Part print with two shaded views. Sizes in mm from the minimum x, y, z corner. A direction names the side the tool comes from. Coordinates: 2 decimals unless noted, no trailing zeros. Loops run counter-clockwise (first coordinate to the right, second up) from the corner with the lowest first, then second, coordinate; pieces in that order, holes last. Notation, with made-up numbers: M -37.75,-23.75 L 2.25,-23.75 A23 cw 2.25,6.25 Z; hole C 17,15 d4. An arc over 180 degrees is marked long. Use CSV: the item, a comma, the result in double quotes. Start each with the question number.
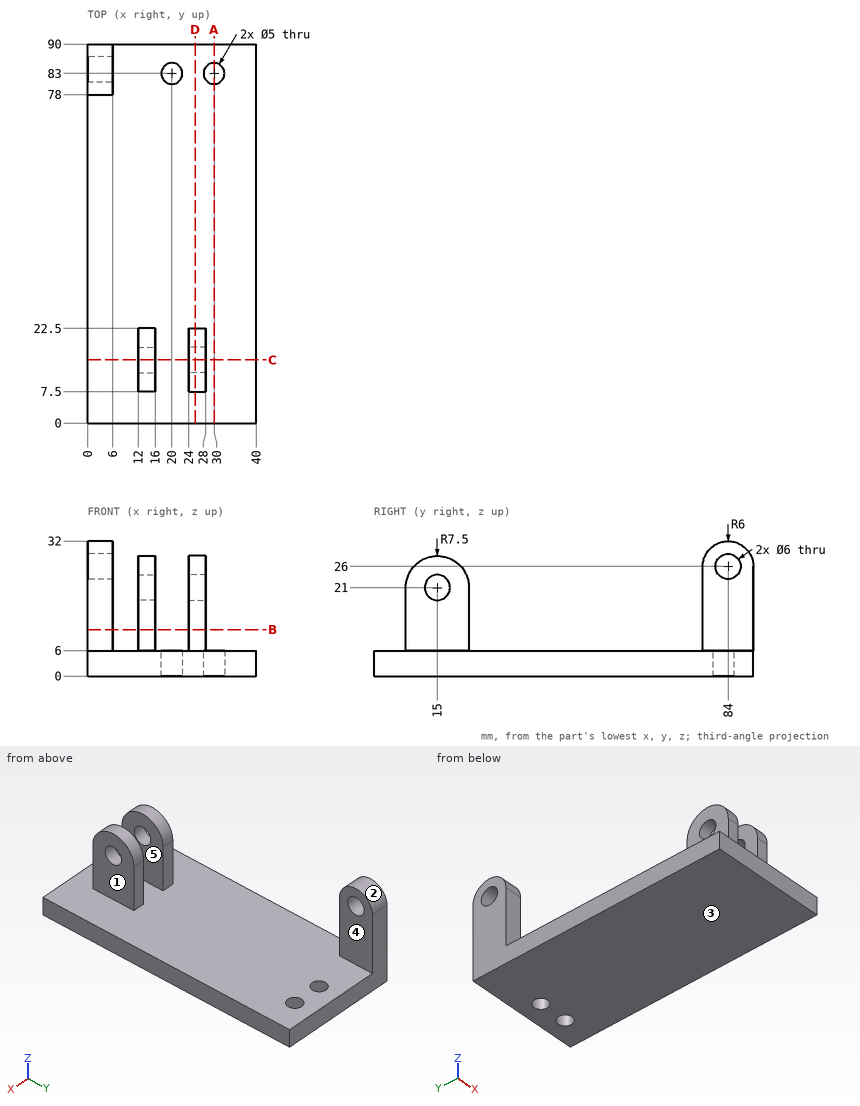
1. Wall check: probe 1 along Y at (x, z) = (30, 3.8); probe 2 along Y at (x, z) = (25.95, 21); probe 3 along Z at (x, y) = (17, 15). Give the ranges that are in metal, low to high.
2. Tool access for the marked faces 1 and 2: list every direction of +Z, -Z, +X, -X, +Y, -Y with a clear straight run to the whole face (end or side of a thin tool).
3. Two-plate mould, pull along X, no slides. Class the marked faces 3, 4 and 5: pulls with the +X half, pulls with the -X half, needs draft (parallel to the pull), parting line crosses it, or undercut.
4. Slice it at D-D, the plane x = 25.5. List the corners of the cut face in (y, z), and give its area (3 significant figures).
5. Slice it at B-B, the plane z = 11. List the corners of the cut face in (x, y), and give its area (3 significant figures).
6. Slice it at A-A, the plane x = 30. List the corners of the cut face in (y, z).
7. Slice it at C-C, the plane y = 15. List the corners of the cut face in (x, z), and give its area (3 significant figures).
8. Pin check, flat tips, straight feed: pin 1 (8 mm diameter, centred on x = 20, y = 83, fed in from +Z); pin 2 (9.5 mm diameter, centred on y = 86, z = 16.5, fed in from +X); pin 3 (7.5 mm diameter, centred on y = 12, z = 18.5, fed in from +X). Stop position of each tip, or through.
Found:
1,probe 1,"0 to 80.5, 85.5 to 90"
1,probe 2,"7.5 to 12, 18 to 22.5"
1,probe 3,"0 to 6"
2,face 1,"+Z, +X, +Y, -Y"
2,face 2,"+Z, +X, -X"
3,face 3,"needs draft"
3,face 4,"pulls with the +X half"
3,face 5,"undercut"
4,outline,"M 0,0 L 90,0 L 90,6 L 22.5,6 L 22.5,21 A7.5 ccw 7.5,21 L 7.5,6 L 0,6 Z; hole C 15,21 d6"
4,area,"825 mm^2"
5,outline,"M 0,78 L 6,78 L 6,90 L 0,90 Z; M 12,7.5 L 16,7.5 L 16,22.5 L 12,22.5 Z; M 24,7.5 L 28,7.5 L 28,22.5 L 24,22.5 Z"
5,area,"192 mm^2"
6,outline,"M 0,0 L 80.5,0 L 80.5,6 L 0,6 Z; M 85.5,0 L 90,0 L 90,6 L 85.5,6 Z"
7,outline,"M 0,0 L 40,0 L 40,6 L 28,6 L 28,18 L 24,18 L 24,6 L 16,6 L 16,18 L 12,18 L 12,6 L 0,6 Z; M 12,24 L 16,24 L 16,28.5 L 12,28.5 Z; M 24,24 L 28,24 L 28,28.5 L 24,28.5 Z"
7,area,"372 mm^2"
8,pin 1,"z = 6"
8,pin 2,"x = 6"
8,pin 3,"x = 28"
